Geometry check sheet. Reference: drawing and pictorial views, mm from the part's lowest x, y, z. Give positions to 0.01 mm unless a question says otherwise; leave off trailing zeros. Write each loop counter-clockwise with the first axis right and the second up, starting at its lowest first coordinate (ties: lowest second). Pieces come first, ordered by that corner, then holes. Notation, with made-up numbers: (-22, -14) - (-6, -14) arc R32 cw to (-6, 13) - close; hole circle Ø2 at (64.5, -15.75). An arc over 180 degrees is marked (long way). Write item = value, one per line. Start each with the question number.
(1) Section check B-B, the plane z = 9. Enter the section's corners in (x, y), plus the area to 3 significant figures.
(2) Section check A-A, the plane x = 35. Enter the section's corners in (y, z), plus the area to 3 significant figures.
(3) Draft check along Z on the marked faces 1, 2 and 3. Enter one of: pulls with the +Z half, pulls with the -Z half, needs draft (parallel to the pull), parting line crosses it, or undercut.
(4) Section check C-C, the plane y = 4.2. Enter the section's corners in (x, z), plus the area to 3 significant figures.
(5) Thickness scan on L1, parallel to X at y = 2.4, z = 9; L2, parallel to Z at x = 35, y = 1.55; L3, parallel to X at y = 2.55, z = 10.5. Record the ranges inside material, lowest first.
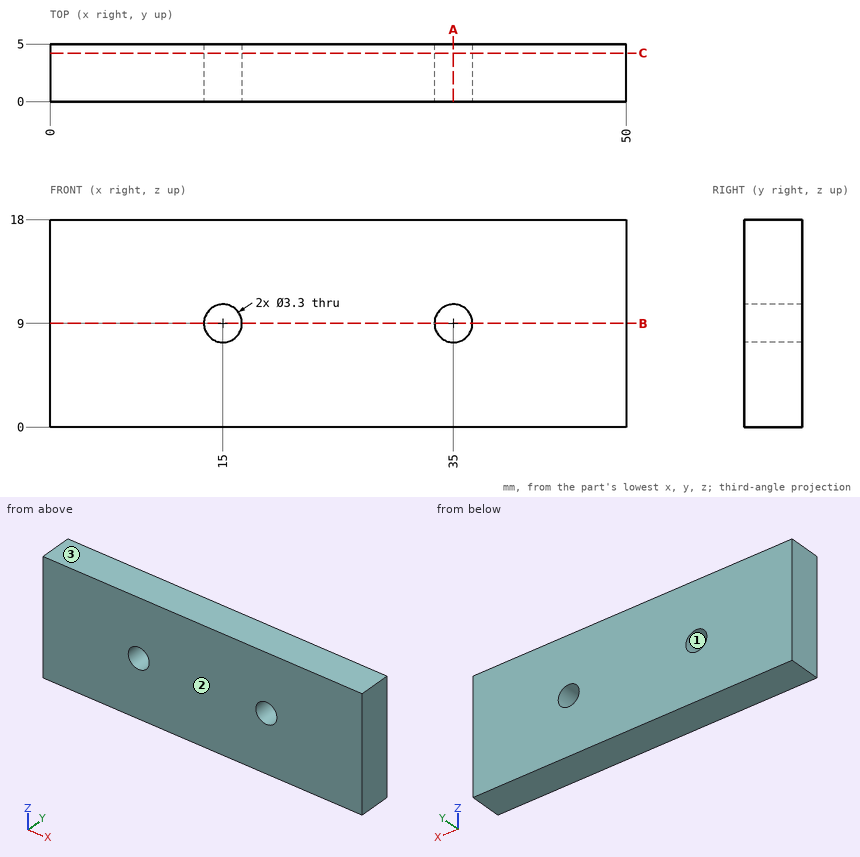
Model answer:
q1.outline = (0, 0) - (13.35, 0) - (13.35, 5) - (0, 5) - close; (16.65, 0) - (33.35, 0) - (33.35, 5) - (16.65, 5) - close; (36.65, 0) - (50, 0) - (50, 5) - (36.65, 5) - close
q1.area = 217 mm²
q2.outline = (0, 0) - (5, 0) - (5, 7.35) - (0, 7.35) - close; (0, 10.65) - (5, 10.65) - (5, 18) - (0, 18) - close
q2.area = 73.5 mm²
q3.face_1 = undercut
q3.face_2 = needs draft
q3.face_3 = pulls with the +Z half
q4.outline = (0, 0) - (50, 0) - (50, 18) - (0, 18) - close; hole circle Ø3.3 at (15, 9); hole circle Ø3.3 at (35, 9)
q4.area = 883 mm²
q5.L1 = 0 to 13.35, 16.65 to 33.35, 36.65 to 50
q5.L2 = 0 to 7.35, 10.65 to 18
q5.L3 = 0 to 14.31, 15.69 to 34.31, 35.69 to 50
